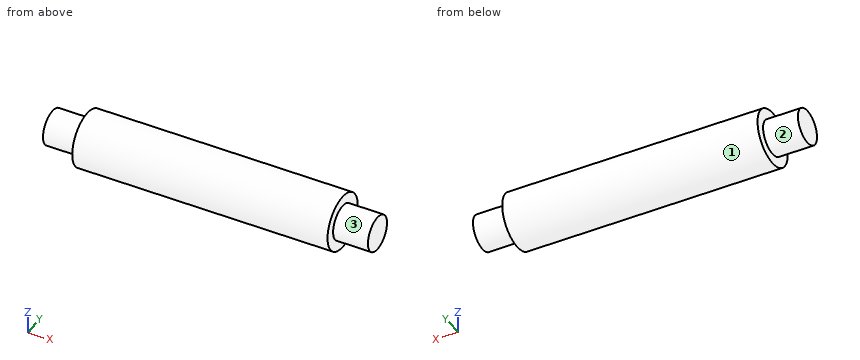
```python
from build123d import *


with BuildPart() as part:
    # Roller Profile Sketch → Roller Body Thin Revolve (revolve)
    with BuildSketch(Plane.XY, mode=Mode.PRIVATE) as roller_body_thin_revolve_sk:
        Polygon((280, 0), (280, 30), (220, 30), (220, 47.5), (-220, 47.5), (-220, 30), (-280, 30), (-280, 0), (-270, 0), (-270, 20), (-210, 20), (-210, 37.5), (210, 37.5), (210, 20), (270, 20), (270, 0), align=None)
    revolve(roller_body_thin_revolve_sk.sketch.rotate(Axis((-409.616293783, 0, 0), (1, 0, 0)), 90), axis=Axis((-409.616293783, 0, 0), (1, 0, 0)))


solid = part.part
```
CAD build for the part. Positions are in the model's coordinates, mm. Face numbers are marked on the shaded views. A direction names the side the tool comes from. Coordinates: 2 decimals unless noted, no trailing zeros. Order: outer loops, then holes, each group sorted by start corner. A loop starts at its lowest first (then second) coordinate and runs counter-clockwise, first axis right, second up. Notation, with made-up numbers: M 77,44 L 122,44 A30 ccw 122,77 Z; hole C 54.5,56.25 d2. An arc over 180 degrees is marked long. Write each question's results on one line, items separated by ' | '. Start each with the question number.
Q1. Flat gauge pins, fed straight in: P1, Ø10, axis at x = -214.5, z = -37, coming from the +Y side; P2, Ø5, axis at x = 80, z = 24, coming from the +Y side; P3, Ø1, axis at x = -181.5, y = 34.5, coming from the -Z side. Where does each tip first touch, or does it go through?
Q2. Cut at C-C (x = 242). List the corners of the cut face in (y, z), then the cut area to 3 significant figures.
Q3. Which spindle directions (+Z, -Z, +X, -X, +Y, -Y) get a long thin tool onto all of the face, cutting with end or side? Do the marked faces 1, 2 and 3. Say none if no direction does.
Q4. Drill centre lines: probe 1 along X at (y, z) = (36.5, -6.5); probe 2 along X at (y, z) = (-22, 19.5); probe 3 along Y at (x, z) = (15, 0). Where is each one in solid material? Low to high. Write a range as from..to.
Q5. Cut at D-D (x = -35.5). List the corners of the cut face in (y, z), then the cut area to 3 significant figures.
Q6. Cut at A-A (y = 0). List the corners of the cut face in (x, z), then the cut area to 3 significant figures.
Found:
1) P1: y = 35.1 | P2: y = 42.36 | P3: z = -33.17
2) outline: C 0,0 d60; hole C 0,0 d40 | area: 1,570 mm²
3) face 1: +X, -X | face 2: -X | face 3: +X
4) probe 1: -220..-210, 210..220 | probe 2: -280..-210, 210..280 | probe 3: -47.5..-37.5, 37.5..47.5
5) outline: C 0,0 d95; hole C 0,0 d75 | area: 2,670 mm²
6) outline: M -280,-30 L -220,-30 L -220,-47.5 L 220,-47.5 L 220,-30 L 280,-30 L 280,30 L 220,30 L 220,47.5 L -220,47.5 L -220,30 L -280,30 Z; hole M -270,-20 L -210,-20 L -210,-37.5 L 210,-37.5 L 210,-20 L 270,-20 L 270,20 L 210,20 L 210,37.5 L -210,37.5 L -210,20 L -270,20 Z | area: 12,700 mm²
